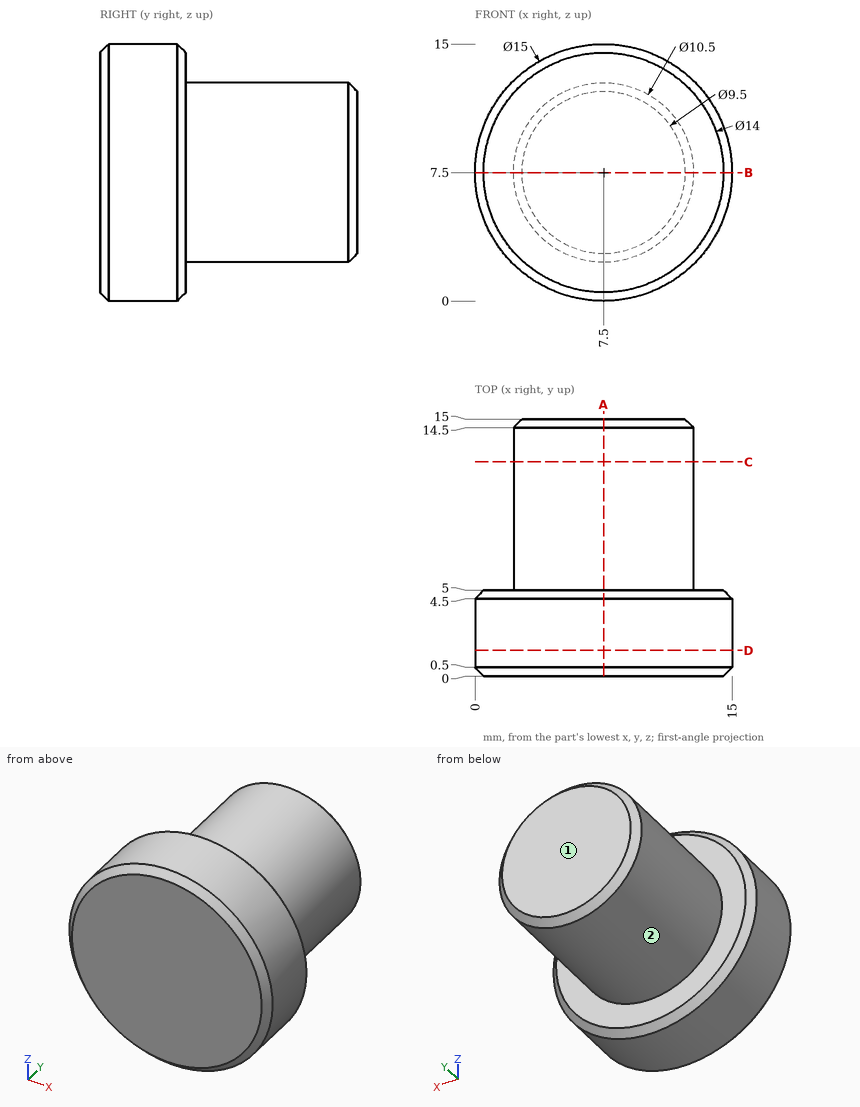
Here's the drawing with two shaded views (mm, measured from the low corner). I have some questions. A direction names the side the tool comes from. Give positions to 0.01 mm unless a question says otherwise; leave off trailing zeros. Order: outer loops, then holes, each group sorted by start corner. A loop starts at its lowest first (then second) coordinate and runs counter-clockwise, first axis right, second up.
Q1. Suppose I cut it at C-C, the plane y = 12.5. Write out the boundary of the cut face in (x, z).
Q2. Suppose I cut it at D-D, the plane y = 1.5. Write out the boundary of the cut face in (x, z).
Q3. Suppose I cut it at B-B, the plane z = 7.5. Write out the boundary of the cut face in (x, y).
Q4. For the marked faces 1 and 2, which set-ups out of +Z, -Z, +X, -X, +Y, -Y let a thin tool reach every point of the face, with its end or its side?
Q5. I'm going to push flat-ended pins straight in: P1, Ø1.5, axis at x = 13.5, z = 6, coming from the +Y side; P2, Ø2, axis at y = 2.5, z = 11.5, coming from the -X side; P3, Ø3, axis at x = 5.5, y = 13, coming from the +Z side; P4, Ø8, axis at y = 3, z = 8.5, coming from the -X side. Where does each tip first touch, or does it pass through?
Q6. Suppose I cut it at A-A, the plane x = 7.5. Write out the boundary of the cut face in (y, z), and give its area (3 significant figures).
Q7. If I drill on line 1 along Y through (x, z) = (2.25, 9.75); line 2 along X through (y, z) = (2, 4); line 3 along X through (y, z) = (4, 6.75), over which ranges is the centre line in solid material (lowest first)?
Solution:
1. outline: circle Ø10.5 at (7.5, 7.5)
2. outline: circle Ø15 at (7.5, 7.5)
3. outline: (0, 0.5) - (0.5, 0) - (14.5, 0) - (15, 0.5) - (15, 4.5) - (14.5, 5) - (12.75, 5) - (12.75, 14.5) - (12.25, 15) - (2.75, 15) - (2.25, 14.5) - (2.25, 5) - (0.5, 5) - (0, 4.5) - close
4. face 1: +Z, -Z, +X, -X, +Y
4. face 2: +Y
5. P1: stops at y = 5
5. P2: stops at x = 0.63
5. P3: stops at z = 12.73
5. P4: stops at x = 0
6. outline: (0, 0.5) - (0.5, 0) - (4.5, 0) - (5, 0.5) - (5, 2.25) - (14.5, 2.25) - (15, 2.75) - (15, 12.25) - (14.5, 12.75) - (5, 12.75) - (5, 14.5) - (4.5, 15) - (0.5, 15) - (0, 14.5) - close
6. area: 179 mm2
7. line 1: y = 0 to 5
7. line 2: x = 0.87 to 14.13
7. line 3: x = 0.04 to 14.96
